```python
from build123d import *

# Parameters (mm, degrees)
SKETCH_1_R          = 17.25
EXTRUDE_1_DEPTH     = 10
SKETCH_2_R          = 17.5
CUT_EXTRUDE_1_DEPTH = 10


with BuildPart() as part:
    # 草图1 → 凸台-拉伸1 (new body)
    with BuildSketch(Plane(origin=(0, 0, 0), x_dir=(1, 0, 0), z_dir=(0, 1, 0))):
        with BuildLine():
            Line((0, 0), (160, 0))
            Line((160, 0), (108.961672936, 104.187459277))
            ThreePointArc((108.961672936, 104.187459277), (80, 122.25), (51.038327064, 104.187459277))
            Line((51.038327064, 104.187459277), (0, 0))
        make_face()
        with Locations(Location((80, 90, 0), (0, 0, 270))):
            Circle(SKETCH_1_R, mode=Mode.SUBTRACT)
    extrude(amount=EXTRUDE_1_DEPTH)

    # 草图2 → 切除-拉伸1 (cut)
    with BuildSketch(Plane(origin=(0, 10, 0), x_dir=(1, 0, 0), z_dir=(0, 1, 0))):
        with Locations(Location((80, 90, 0), (0, 0, 270))):
            Circle(SKETCH_2_R)
    extrude(amount=-CUT_EXTRUDE_1_DEPTH, mode=Mode.SUBTRACT)


solid = part.part
```
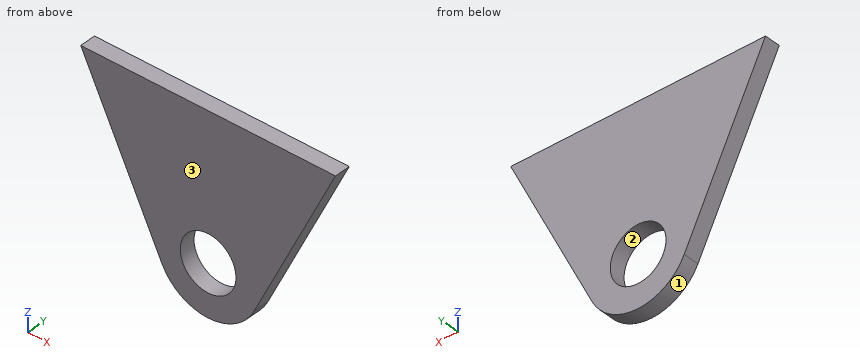
Build history of the part. All positions in model axes, mm. Face numbers are marked on the shaded views. Give positions to 0.01 mm unless a question says otherwise; leave off trailing zeros. Order: outer loops, then holes, each group sorted by start corner. A loop starts at its lowest first (then second) coordinate and runs counter-clockwise, first axis right, second up. Notation, with made-up numbers: M 52,-11 L 75,-11 A20 ccw 75,14 Z; hole C 15.5,32.25 d8. An arc over 180 degrees is marked long. Write item = value, one per line. Start each with the question number.
(1) Pin check, flat tips, straight feed: pin 1 Ø2 at (x, y) = (33, 7) entering from -Z; pin 2 Ø4 at (y, z) = (7.5, -97.5) entering from +X; pin 3 Ø1.5 at (y, z) = (5, -87) entering from -X; pin 4 Ø4 at (x, z) = (121, -85.5) entering from +Y. Stop position of each tip, or through.
(2) Slice it at A-A on x = 80. Write the cut outline in (y, z).
(3) Slice it at D-D on x = 115.5. Write the cut outline in (y, z), plus the area to 3 significant figures.
(4) Slice it at C-C on z = -90. Write the cut outline in (x, y), plus the area to 3 significant figures.
(5) Two-plate mould, pull along Z, no slides. Class the marked faces 1, 2 and 3: released by +Z, released by -Z, zero draft, split by the parting line, or undercut.
(6) Probe L1, parallel to Z at x = 74, y = 5.75; L2, parallel to X at y = 4.25, z = -90; L3, parallel to X at y = 1.5, z = -94. List the from-to ranges inside material, lowest first. Write a range as [from, to].
(7) Slice it at B-B on y = 6.75. Write the cut outline in (x, z), plus the area to 3 significant figures.
Responses:
q1.pin_1 = -69.41
q1.pin_2 = 113.22
q1.pin_3 = 42.25
q1.pin_4 = through
q2.outline = M 0,-122.25 L 10,-122.25 L 10,-107.5 L 0,-107.5 Z; M 0,-72.5 L 10,-72.5 L 10,0 L 0,0 Z
q3.outline = M 0,-90.84 L 10,-90.84 L 10,0 L 0,0 Z
q3.area = 908 mm2
q4.outline = M 44.09,0 L 62.5,0 L 62.5,10 L 44.09,10 Z; M 97.5,0 L 115.91,0 L 115.91,10 L 97.5,10 Z
q4.area = 368 mm2
q5.face_1 = released by -Z
q5.face_2 = undercut
q5.face_3 = zero draft
q6.L1 = [-121.69, -106.44], [-73.56, 0]
q6.L2 = [44.09, 62.5], [97.5, 115.91]
q6.L3 = [46.05, 62.96], [97.04, 113.95]
q7.outline = M 0,0 L 51.04,-104.19 A32.25 ccw 108.96,-104.19 L 160,0 Z; hole C 80,-90 d35
q7.area = 11,100 mm2
